The listing builds one solid part. Answer for the finished solid, in the listing's coordinates (mm). A direction names the side the tool comes from. Coordinates: 2 decimals unless noted, no trailing zeros. Loops run counter-clockwise (first coordinate to the right, second up) from the corner with the lowest first, then second, coordinate; pieces in that order, holes last. Notation, with made-up numbers: (-5, -27.75) - (16, -27.75) arc R17 cw to (16, 4.25) - close; hole circle Ø5 at (31, 59). An arc over 180 degrees is marked (long way). Put each result on its own line as item: value.
```python
from build123d import *

# Parameters (mm, degrees)
SKETCH_1_R               = 30
EXTRUDE_1_DEPTH          = 122
CUT_EXTRUDE_START        = -12
SKETCH_2_OUTSIDE_W       = 91.722
SKETCH_2_OUTSIDE_H       = 91.722
SKETCH_2_OUTSIDE_R       = 12.5
CUT_EXTRUDE_1_DEPTH      = 118.16655914
HOLE_WIZARD_M6_1_D       = 6.6
SKETCH_7_R               = 16
EXTRUDE_3_DEPTH          = 4
MM_0_D                   = 4
HOLE_WIZARD_M6_1_2_D     = 5
HOLE_WIZARD_M6_1_2_DEPTH = 15
HOLE_WIZARD_M6_1_2_TIP   = 1.502151548


with BuildPart() as part:
    # 草图1 → 凸台-拉伸1 (new body)
    with BuildSketch(Plane(origin=(0, 0, 0), x_dir=(1, 0, 0), z_dir=(0, 1, 0))):
        with Locations(Location((0, 0, 0), (0, 0, 90))):
            Circle(SKETCH_1_R)
    extrude(amount=EXTRUDE_1_DEPTH)

    # 草图2 outside → 切除-拉伸1 (cut, through all)
    with BuildSketch(Plane(origin=(0, 122, 0), x_dir=(1, 0, 0), z_dir=(0, 1, 0)).offset(CUT_EXTRUDE_START)):
        Rectangle(SKETCH_2_OUTSIDE_W, SKETCH_2_OUTSIDE_H)
        with Locations(Location((0, 0, 0), (0, 0, 270))):
            Circle(SKETCH_2_OUTSIDE_R, mode=Mode.SUBTRACT)
    extrude(amount=-CUT_EXTRUDE_1_DEPTH, mode=Mode.SUBTRACT)

    # Hole Wizard M6 _1 (through all)
    with Locations(Plane(origin=(0, 110, 0), x_dir=(-1, 0, 0), z_dir=(0, -1, 0))):
        with Locations((-24, 0), (-16.970562748, 16.970562748), (0, 24), (16.970562748, 16.970562748), (24, 0), (16.970562748, -16.970562748), (0, -24), (-16.970562748, -16.970562748)):
            Hole(HOLE_WIZARD_M6_1_D / 2)

    # 草图7 → 凸台-拉伸3 (add)
    with BuildSketch(Plane(origin=(0, 122, 0), x_dir=(1, 0, 0), z_dir=(0, 1, 0))):
        with Locations(Location((0, 0, 0), (0, 0, 270))):
            Circle(SKETCH_7_R)
    extrude(amount=EXTRUDE_3_DEPTH)

    # 大小mm 暗销孔0 (through all)
    with Locations(Plane(origin=(0, 110, 0), x_dir=(-1, 0, 0), z_dir=(0, -1, 0))):
        with Locations((-9.184402377, 22.17310878)):
            Hole(MM_0_D / 2)

    # Hole Wizard M6 _1 2
    with Locations(Plane(origin=(0, 0, 0), x_dir=(-1, 0, 0), z_dir=(0, -1, 0))):
        with Locations((0, 0)):
            Hole(HOLE_WIZARD_M6_1_2_D / 2, depth=HOLE_WIZARD_M6_1_2_DEPTH)
            with Locations((0, 0, -(HOLE_WIZARD_M6_1_2_DEPTH + HOLE_WIZARD_M6_1_2_TIP / 2))):  # 118° drill point
                Cone(0, HOLE_WIZARD_M6_1_2_D / 2, HOLE_WIZARD_M6_1_2_TIP, mode=Mode.SUBTRACT)


solid = part.part
```
1) The part is cut by section D-D (z = 6). Give the vertices of the cut face in (x, y).
Found:
outline: (-29.39, 110) - (-10.97, 110) - (-10.97, 0) - (10.97, 0) - (10.97, 110) - (29.39, 110) - (29.39, 122) - (14.83, 122) - (14.83, 126) - (-14.83, 126) - (-14.83, 122) - (-29.39, 122) - close
2) For faces 1 (the face through (-15.62, 123.97, -3.47)), 2 (the face through (3.755, 55.77, 11.923)), 3 (the face through (27.05, 116.08, 1.26)), determine the directions among +Z, -Z, +X, -X, +Y, -Y from which every point of the face is accessible in a straight line to the end or side of a thin tool.
Found:
face 1: +Y
face 2: -Y
face 3: +Y, -Y
3) Each of these flat-tipped pins is pushed along its axis until it touches: pin 1 (8 mm diameter, centred on x = 16, z = 8, fed in from +Y); pin 2 (4.5 mm diameter, centred on x = 9.18, z = -22.17, fed in from -Y); pin 3 (7.5 mm diameter, centred on x = 16.97, z = -16.97, fed in from +Y); pin 4 (4 mm diameter, centred on x = -10, y = 74.5, fed in from -Z). Where does it stop, or does it pass through?
Found:
pin 1: stops at y = 126
pin 2: stops at y = 110
pin 3: stops at y = 122
pin 4: stops at z = -9.6
4) The part is cut by section B-B (y = 60). Give the vertices of the cut face in (x, z).
Found:
outline: circle Ø25 at (0, 0)
5) For a pull along X with two mould halves and no side action, classify faces 4 (the face through (-1.32, 115.92, 29.97)), 5 (the face through (-0.72, 116.08, -20.78)), 6 (the face through (0, 110, 13)), 7 (the face through (8.75, 116.08, -20.22)) as pulls with the +X half, pulls with the -X half, needs draft (parallel to the pull), parting line crosses it, or undercut.
Found:
face 4: parting line crosses it
face 5: undercut
face 6: needs draft
face 7: undercut
6) The part is cut by section A-A (x = -24). Give the vertices of the cut face in (y, z), and give its area (3 significant figures).
Found:
outline: (110, -18) - (122, -18) - (122, -3.3) - (110, -3.3) - close; (110, 3.3) - (122, 3.3) - (122, 18) - (110, 18) - close
area: 353 mm^2
7) Straight lines are drawn through the part: L1, parallel to Y at x = -20.5, z = -21; L2, parallel to Y at x = 14, z = 2; L3, parallel to Z at x = 26.5, y = 120. For each, find the intervals that lie inside material, in ascending order. Write a range as [from, to].
Found:
L1: y = [110, 122]
L2: y = [110, 126]
L3: z = [-14.06, -2.15], [2.15, 14.06]
8) The part is cut by section C-C (x = -9.5). Give the vertices of the cut face in (y, z), and give its area (3 significant figures).
Found:
outline: (0, -8.12) - (110, -8.12) - (110, -28.46) - (122, -28.46) - (122, -12.87) - (126, -12.87) - (126, 12.87) - (122, 12.87) - (122, 28.46) - (110, 28.46) - (110, 8.12) - (0, 8.12) - close
area: 2,570 mm^2
